Could you check a few things on this model? Use its own coordinates, in mm. Face numbers are marked on the shaded views. A direction names the side the tool comes from. Round coordinates to 2 decimals unless told otherwise and drop trailing zeros. Loops run counter-clockwise (first coordinate to the right, second up) from the corner with the lowest first, then second, coordinate; pieces in that order, holes last. Notation, with made-up numbers: M -27,78 L 20,78 A21 ccw 20,104 Z; hole C 83,33.25 d11. An arc over 180 degrees is marked long. Answer in a Markdown table with one row per item.
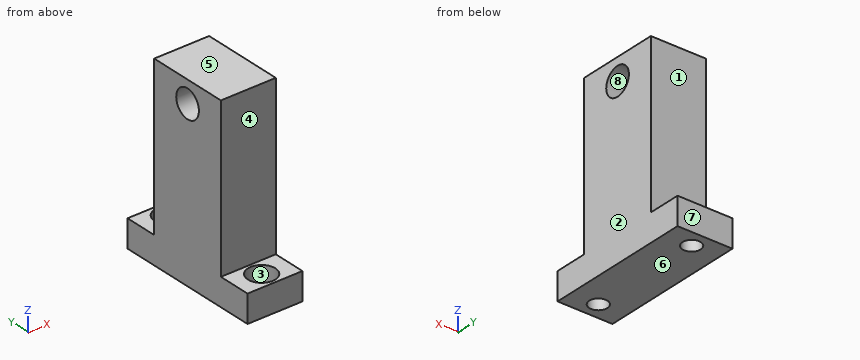
```python
from build123d import *

# Parameters (mm, degrees)
SKETCH1_W                               = 20
SKETCH1_H                               = 54
BOSS_EXTRUDE1_DEPTH                     = 10
SKETCH2_W                               = 20
SKETCH2_H                               = 30
BOSS_EXTRUDE2_DEPTH                     = 58
CBORE_FOR_M6_HEX_HEAD_BOLT1_D           = 6.6
CBORE_FOR_M6_HEX_HEAD_BOLT1_CBORE_D     = 10
CBORE_FOR_M6_HEX_HEAD_BOLT1_CBORE_DEPTH = 6
M12_TAPPED_HOLE1_D                      = 10.2


with BuildPart() as part:
    # Sketch1 → Boss-Extrude1 (new body)
    with BuildSketch(Plane.XY):
        with Locations((-26.388136882, 2.617870722)):
            Rectangle(SKETCH1_W, SKETCH1_H)
    extrude(amount=BOSS_EXTRUDE1_DEPTH)

    # Sketch2 → Boss-Extrude2 (add)
    with BuildSketch(Plane.XY.offset(10)):
        with Locations((-26.388136882, 2.617870722)):
            Rectangle(SKETCH2_W, SKETCH2_H)
    extrude(amount=BOSS_EXTRUDE2_DEPTH)

    # CBORE for M6 Hex Head Bolt1 (through all)
    with Locations(Plane.XY.offset(10)):
        with Locations((-26.388136882, 23.617870722), (-26.388136882, -18.382129278)):
            CounterBoreHole(CBORE_FOR_M6_HEX_HEAD_BOLT1_D / 2, CBORE_FOR_M6_HEX_HEAD_BOLT1_CBORE_D / 2, CBORE_FOR_M6_HEX_HEAD_BOLT1_CBORE_DEPTH)

    # M12 Tapped Hole1 (through all)
    with Locations(Plane.ZY.offset(36.388136882)):
        with Locations((60, 2.617870722)):
            Hole(M12_TAPPED_HOLE1_D / 2)


solid = part.part
```
1) I want a section at C-C, the plane y = 4. Please give me the cut outline in (x, z), plus the area to 3 significant figures.
Computed:
| item | result |
|---|---|
| outline | M -36.39,0 L -16.39,0 L -16.39,55.09 L -36.39,55.09 Z; M -36.39,64.91 L -16.39,64.91 L -16.39,68 L -36.39,68 Z |
| area | 1,160 mm² |
2) If we mould it in two halves opening along Z, with no side actions, what happens to the marked faces 5, 6, 7 and 8? For each: released by +Z, released by -Z, zero draft, split by the parting line, or undercut.
Computed:
| item | result |
|---|---|
| face 5 | released by +Z |
| face 6 | released by -Z |
| face 7 | zero draft |
| face 8 | undercut |
3) I need wall thicknesses on line 1 (Y direction, x = -23.5, z = 60); line 2 (Z direction, x = -18, y = 23); line 3 (Z direction, x = -23.25, y = 26). Which ranges of each line are inside material? Lowest first, please.
Computed:
| item | result |
|---|---|
| line 1 | y = -12.38 to -2.48, 7.72 to 17.62 |
| line 2 | z = 0 to 10 |
| line 3 | z = 0 to 4 |
4) I want a section at D-D, the plane x = -19. Please give me the cut outline in (y, z).
Computed:
| item | result |
|---|---|
| outline | M -24.38,0 L 29.62,0 L 29.62,10 L 17.62,10 L 17.62,68 L -12.38,68 L -12.38,10 L -24.38,10 Z; hole C 2.62,60 d10.2 |
5) I want a section at B-B, the plane x = -26.5. Please give me the cut outline in (y, z), plus the area to 3 significant figures.
Computed:
| item | result |
|---|---|
| outline | M -24.38,0 L -21.68,0 L -21.68,4 L -23.38,4 L -23.38,10 L -24.38,10 Z; M -15.08,0 L 20.32,0 L 20.32,4 L 18.62,4 L 18.62,10 L 17.62,10 L 17.62,68 L -12.38,68 L -12.38,10 L -13.38,10 L -13.38,4 L -15.08,4 Z; M 26.92,0 L 29.62,0 L 29.62,10 L 28.62,10 L 28.62,4 L 26.92,4 Z; hole C 2.62,60 d10.2 |
| area | 2,030 mm² |
6) I want a section at A-A, the plane z = 60. Please give me the cut outline in (x, y), plus the area to 3 significant figures.
Computed:
| item | result |
|---|---|
| outline | M -36.39,-12.38 L -16.39,-12.38 L -16.39,-2.48 L -36.39,-2.48 Z; M -36.39,7.72 L -16.39,7.72 L -16.39,17.62 L -36.39,17.62 Z |
| area | 396 mm² |
7) Which directions (+Z, -Z, +X, -X, +Y, -Y) give clear straight access to the entire face, cutting with the end or side of a thin tool? Please do the marked faces 1, 2, 3 and 4.
Computed:
| item | result |
|---|---|
| face 1 | +Z, +X, -X, +Y |
| face 2 | +Z, -Z, +X, +Y, -Y |
| face 3 | +Z |
| face 4 | +Z, +X, -X, -Y |
8) Will these pins go through, and if not, where does the flat tip stop? P1, Ø6, axis at x = -26.5, z = 40, coming from the +Y side; P2, Ø8, axis at x = -27.5, y = -18.5, coming from the +Z side; P3, Ø5.5, axis at x = -26.39, y = -18.38, coming from the +Z side; P4, Ø5, axis at x = -30.5, y = -17, coming from the -Z side.
Computed:
| item | result |
|---|---|
| P1 | stops at y = 17.62 |
| P2 | stops at z = 10 |
| P3 | passes through |
| P4 | stops at z = 0 |
